The drawing under review shows one solid part. Ordinate dimensions are in mm from its lowest x, y, z. A direction names the side the tool comes from. Coordinates: 2 decimals unless noted, no trailing zeros. Order: outer loops, then holes, each group sorted by start corner. A loop starts at its lowest first (then second) coordinate and runs counter-clockwise, first axis right, second up. Notation, with made-up numbers: (69.5, -13.75) -> (94.5, -13.75) arc R16 ccw to (94.5, 9.25) -> close; hole circle Ø2 at (62, 1). An arc over 180 degrees is marked (long way). Put each result on its own line as item: value.
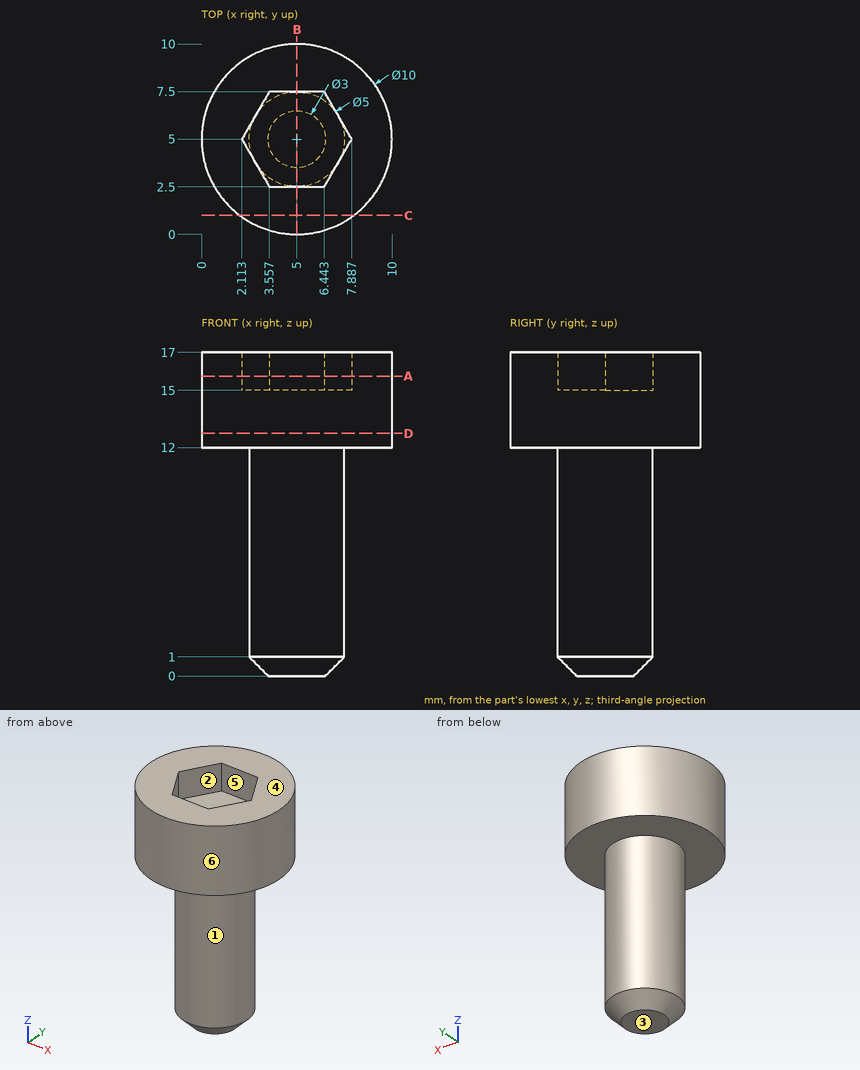
Item 1: Consider section C-C on y = 1. Write out the cut boundary in (x, z), and give its area (3 significant figures).
Answers below:
outline: (2, 12) -> (8, 12) -> (8, 17) -> (2, 17) -> close
area: 30.0 mm^2
Item 2: For the marked faces 1, 2 and 3, list the 3-axis set-ups (+Z, -Z, +X, -X, +Y, -Y) from which the entire face can be reached by the end or side of a thin tool; tool diameter is ignored.
Answers below:
face 1: -Z
face 2: +Z
face 3: -Z, +X, -X, +Y, -Y
Item 3: Mouldability with a two-part tool opening along Y and no side actions: class the marked faces 4, 5 and 6 as +Y half, -Y half, draft (parallel to the pull), parting line (faces both ways), or undercut.
Answers below:
face 4: draft
face 5: undercut
face 6: parting line
Item 4: Consider section D-D on z = 12.75. Write out the cut boundary in (x, y).
Answers below:
outline: circle Ø10 at (5, 5)
Item 5: Consider section B-B on x = 5. Write out the cut boundary in (y, z), and give its area (3 significant figures).
Answers below:
outline: (0, 12) -> (2.5, 12) -> (2.5, 1) -> (3.5, 0) -> (6.5, 0) -> (7.5, 1) -> (7.5, 12) -> (10, 12) -> (10, 17) -> (7.5, 17) -> (7.5, 15) -> (2.5, 15) -> (2.5, 17) -> (0, 17) -> close
area: 99.0 mm^2
Item 6: For pin 1 Ø5 at (y, z) = (2, 6) entering from -X; pin 2 Ø1.5 at (x, y) = (8.5, 6) entering from -Z; pin 3 Ø1.5 at (x, z) = (2.5, 12.5) entering from -Y, all flat-tipped, find the tip position at first contact; note any pin that passes through.
Answers below:
pin 1: x = 2.55
pin 2: z = 12
pin 3: y = 0.32
Item 7: Consider section A-A on z = 15.75. Write out the cut boundary in (x, y).
Answers below:
outline: circle Ø10 at (5, 5); hole (2.11, 5) -> (3.56, 2.5) -> (6.44, 2.5) -> (7.89, 5) -> (6.44, 7.5) -> (3.56, 7.5) -> close
Item 8: For line 1 (Z direction, x = 6.5, y = 2.5); line 2 (X direction, y = 3, z = 5.5); line 3 (Z direction, x = 5.5, y = 3.75), list the stretches that pass through material, from the lowest coordinate up. Write a range as from..to.
Answers below:
line 1: 12..17
line 2: 3.5..6.5
line 3: 0..15
